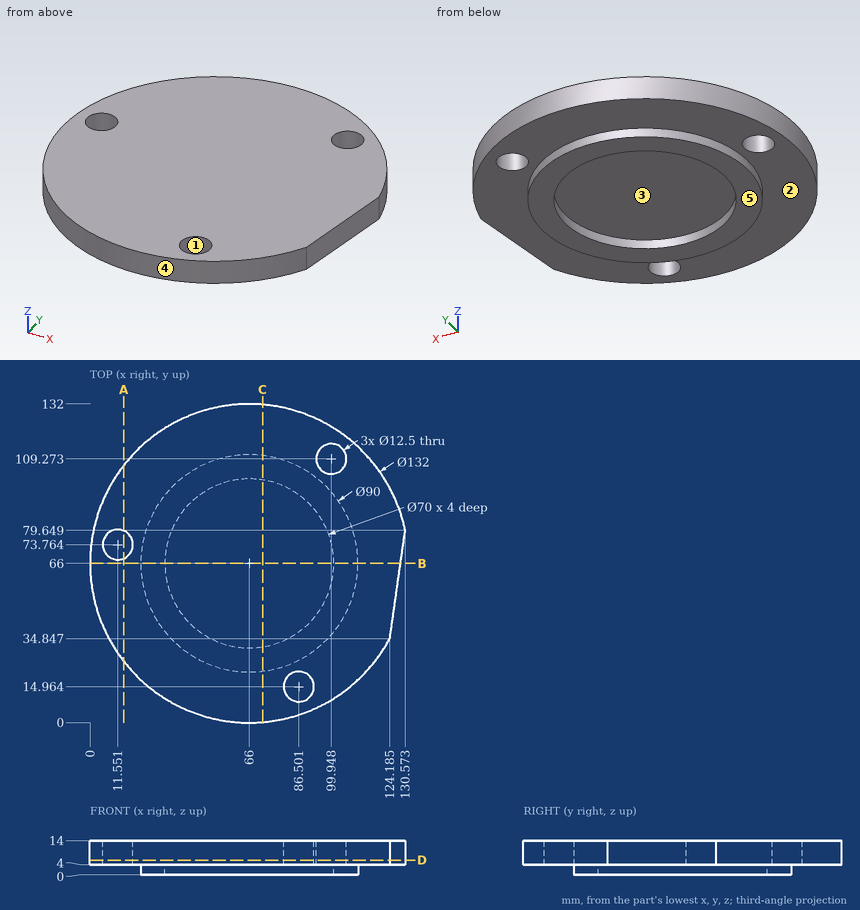
Design review of the part shown in the three views and the two pictorial views. Dimensions are in mm from the part's minimum x, y and z. A direction names the side the tool comes from. Round coordinates to 2 decimals unless told otherwise and drop trailing zeros. Write each loop counter-clockwise with the first axis right and the second up, starting at its lowest first coordinate (ties: lowest second). Pieces come first, ordered by that corner, then holes.
Item 1: For probe 1 along Y at (x, z) = (66, 1.55); probe 2 along Y at (x, z) = (67, 13); probe 3 along Z at (x, y) = (96, 58.5), list the stretches that pass through material, from the lowest coordinate up.
Item 2: We need section D-D on z = 6. State how many separate pieces and enclosed holes the cut face has, and give its area (3 significant figures).
Item 3: For the marked faces 1 and 2, list the 3-axis set-ups (+Z, -Z, +X, -X, +Y, -Y) from which the entire face can be reached by the end or side of a thin tool; tool diameter is ignored.
Item 4: We need section C-C on x = 71.5. Write out the cut boundary in (y, z) (1 decimal), and give its area (3 significant figures).
Item 5: Clearance check with flat-ended pins moving along their axes: pin 1 Ø6 at (y, z) = (69.5, 6) entering from -X; pin 2 Ø5 at (y, z) = (95, 11.5) entering from -X; pin 3 Ø1.5 at (x, y) = (73, 37) entering from -Z; pin 4 Ø11 at (x, y) = (86.5, 14.96) entering from +Z. State where each tip first meets the part, or that it passes through.
Item 6: We need section A-A on x = 14. Write out the cut boundary in (y, z) (1 decimal).
Item 7: We need section B-B on y = 66. Write out the cut boundary in (x, z).
Item 8: The part is to be moulded in two halves that separate along X. For the marked faces 3, 4 and 5, say which applies: +X half, -X half, draft (parallel to the pull), parting line (faces both ways), or undercut.
Returned:
1. probe 1: y = 21 to 31, 101 to 111
1. probe 2: y = 0.01 to 131.99
1. probe 3: z = 4 to 14
2. separate pieces: 1
2. enclosed holes: 3
2. area: 13,200 mm2
3. face 1: +Z, -Z
3. face 2: -Z
4. outline: (0.2, 4) - (21.3, 4) - (21.3, 0) - (31.4, 0) - (31.4, 4) - (100.6, 4) - (100.6, 0) - (110.7, 0) - (110.7, 4) - (131.8, 4) - (131.8, 14) - (0.2, 14) - close
4. area: 1,400 mm2
5. pin 1: stops at x = 0
5. pin 2: stops at x = 5.55
5. pin 3: stops at z = 4
5. pin 4: passes through
6. outline: (25.4, 4) - (68, 4) - (68, 14) - (25.4, 14) - close; (79.5, 4) - (106.6, 4) - (106.6, 14) - (79.5, 14) - close
7. outline: (0, 4) - (21, 4) - (21, 0) - (31, 0) - (31, 4) - (101, 4) - (101, 0) - (111, 0) - (111, 4) - (128.63, 4) - (128.63, 14) - (0, 14) - close
8. face 3: undercut
8. face 4: parting line
8. face 5: draft
